Verification items for the finished model (mm, model axes). Round coordinates to 2 decimals unless told otherwise and drop trailing zeros. Loops run counter-clockwise (first coordinate to the right, second up) from the corner with the lowest first, then second, coordinate; pieces in that order, holes last.
from build123d import *

# Parameters (mm, degrees)
SKETCH_1_W         = 60
SKETCH_1_H         = 20
EXTRUDE_1_DEPTH    = 25
HOLE_WIZARD_M6_1_D = 6.6


with BuildPart() as part:
    # 草图1 → 凸台-拉伸1 (new body)
    with BuildSketch(Plane.XY):
        Rectangle(SKETCH_1_W, SKETCH_1_H)
    extrude(amount=EXTRUDE_1_DEPTH)

    # M6 间隙孔1 (through all)
    with Locations(Plane.XY.offset(25)):
        with Locations((-22.5, 0), (22.5, 0)):
            Hole(HOLE_WIZARD_M6_1_D / 2)


solid = part.part
1. Scan lines: L1, parallel to Y at x = 22.5, z = 15.25; L2, parallel to X at y = 0.75, z = 4.25. Record each from-to range of solid material in increasing order.
2. Release check for a two-part mould opening along X. For faces 1 (the face through (19.45, -1.26, 12.33)), 2 (the face through (0, 10, 12)), 3 (the face through (-30, 0, 12)) record: released by +X, released by -X, zero draft, split by the parting line, or undercut.
3. Section check B-B (y = 0). Enter the section's corners in (x, z).
4. Section check A-A (x = -22.5). Enter the section's corners in (y, z), then the cut area to 3 significant figures.
5. Section check C-C (z = 1.75). Enter the section's corners in (x, y).
Taken from the geometry:
1. L1: y = -10 to -3.3, 3.3 to 10
1. L2: x = -30 to -25.71, -19.29 to 19.29, 25.71 to 30
2. face 1: undercut
2. face 2: zero draft
2. face 3: released by -X
3. outline: (-30, 0) - (-25.8, 0) - (-25.8, 25) - (-30, 25) - close; (-19.2, 0) - (19.2, 0) - (19.2, 25) - (-19.2, 25) - close; (25.8, 0) - (30, 0) - (30, 25) - (25.8, 25) - close
4. outline: (-10, 0) - (-3.3, 0) - (-3.3, 25) - (-10, 25) - close; (3.3, 0) - (10, 0) - (10, 25) - (3.3, 25) - close
4. area: 335 mm2
5. outline: (-30, -10) - (30, -10) - (30, 10) - (-30, 10) - close; hole circle Ø6.6 at (-22.5, 0); hole circle Ø6.6 at (22.5, 0)
